Here's how the part is built. I have some questions about the finished solid (model axes, mm). A direction names the side the tool comes from. Give positions to 0.01 mm unless a question says otherwise; leave off trailing zeros. Write each loop counter-clockwise with the first axis right and the second up, starting at its lowest first coordinate (ties: lowest second). Pieces come first, ordered by that corner, then holes. Notation, with made-up numbers: (73, 46.25) - (94, 46.25) arc R22 cw to (94, 77.25) - close; hole circle Ø4 at (-34, 35.25). An arc over 180 degrees is marked (long way). Use a Markdown table: item, result.
```python
from build123d import *

# Parameters (mm, degrees)
PIVOT_HUB_SKETCH_R            = 28
PIVOT_HUB_SKETCH_R_2          = 15
PIVOT_HUB_56_BORE_30_DEPTH    = 40
LINK_ARM_DEPTH                = 24
FORK_SLOT_SKETCH_W            = 63.247521784
FORK_SLOT_SKETCH_H            = 16
FORK_SLOT_16_DEPTH            = 146.327216997
UPRIGHT_BOSS_SKETCH_R         = 16
UPRIGHT_BOSS_SKETCH_R_2       = 8
UPRIGHT_BOSS_32_BORE_16_DEPTH = 40
JUNCTION_PAD_REACH            = 171.706
TRIANGULAR_RELIEF_CUT_DEPTH   = 10


with BuildPart() as part:
    # Pivot Hub Sketch → Pivot Hub Ø56 Bore Ø30 (new, symmetric)
    with BuildSketch(Plane.XY):
        Circle(PIVOT_HUB_SKETCH_R)
        Circle(PIVOT_HUB_SKETCH_R_2, mode=Mode.SUBTRACT)
    extrude(amount=PIVOT_HUB_56_BORE_30_DEPTH, both=True)

    # Link Arm Profile → Link Arm (add, symmetric)
    with BuildSketch(Plane.XY):
        with BuildLine():
            Line((0, 28), (72, 28))
            ThreePointArc((72, 28), (77.656854249, 30.343145751), (80, 36))
            Line((80, 36), (128, 36))
            Line((128, 36), (128, -4))
            Line((128, -4), (100, -4))
            Line((100, -4), (100, 4))
            ThreePointArc((100, 4), (97.656854249, 9.656854249), (92, 12))
            Line((92, 12), (52, 12))
            ThreePointArc((52, 12), (46.343145751, 9.656854249), (44, 4))
            Line((44, 4), (44, -28))
            Line((44, -28), (0, -28))
            ThreePointArc((0, -28), (28, 0), (0, 28))
        make_face()
    extrude(amount=LINK_ARM_DEPTH, both=True)

    # Fork Slot Sketch → Fork Slot 16 (cut, through all)
    with BuildSketch(Plane(origin=(0, 28, 0), x_dir=(1, 0, 0), z_dir=(0, 1, 0))):
        with Locations((-3.623760892, 0)):
            Rectangle(FORK_SLOT_SKETCH_W, FORK_SLOT_SKETCH_H)
    extrude(amount=-FORK_SLOT_16_DEPTH, mode=Mode.SUBTRACT)

    # Upright Boss Sketch → Upright Boss Ø32 Bore Ø16 (add)
    with BuildSketch(Plane(origin=(0, 36, 0), x_dir=(1, 0, 0), z_dir=(0, 1, 0))):
        with Locations((103.942410132, 0)):
            Circle(UPRIGHT_BOSS_SKETCH_R)
        with Locations(Location((103.942410132, 0, 0), (0, 0, 180))):
            Circle(UPRIGHT_BOSS_SKETCH_R_2, mode=Mode.SUBTRACT)
    extrude(amount=UPRIGHT_BOSS_32_BORE_16_DEPTH)

    # Junction Pad Sketch → Junction Pad (add, up to next)
    with BuildSketch(Plane(origin=(0, 76, 0), x_dir=(1, 0, 0), z_dir=(0, 1, 0)), mode=Mode.PRIVATE) as junction_pad_sk1:
        with BuildLine():
            Line((48, 5), (88.743725978, 5))
            ThreePointArc((88.743725978, 5), (87.942410132, 0), (88.743725978, -5))
            Line((88.743725978, -5), (48, -5))
            Line((48, -5), (48, 5))
        make_face()
    junction_pad_tool1 = extrude(junction_pad_sk1.sketch, amount=-JUNCTION_PAD_REACH, mode=Mode.PRIVATE) - part.part
    add(junction_pad_tool1.solids().sort_by_distance((68.104095, 76, 0))[0])

    # Relief Cut Sketch → Triangular Relief Cut (cut)
    with BuildSketch(Plane.XY.offset(5)):
        Polygon((88.743725978, 76), (48, 28), (48, 76), align=None)
    extrude(amount=-TRIANGULAR_RELIEF_CUT_DEPTH, mode=Mode.SUBTRACT)


solid = part.part
```
Item 1: I need wall thicknesses on line 1 along X through (y, z) = (0, -18.5); line 2 along Y through (x, z) = (0, 17.5); line 3 along X through (y, z) = (18, 5). Which ranges of each line are inside material? Lowest first, please. Write a range as [from, to].
Values:
| item | result |
|---|---|
| line 1 | x = [-28, -15], [15, 44], [100, 128] |
| line 2 | y = [-28, -15], [15, 28] |
| line 3 | x = [28, 128] |
Item 2: If we section it at D-D, the plane x = 23: Write out the boundary of the cut face in (y, z).
Values:
| item | result |
|---|---|
| outline | (-28, -24) - (-15.97, -24) - (-15.97, -40) - (15.97, -40) - (15.97, -24) - (28, -24) - (28, -8) - (-28, -8) - close; (-28, 8) - (28, 8) - (28, 24) - (15.97, 24) - (15.97, 40) - (-15.97, 40) - (-15.97, 24) - (-28, 24) - close |
Item 3: For faces 1 (the flat face through (44, -12, 0)), 2 (the flat face through (12, -12, -8)), 3 (the cylindrical face through (-27.973, 1.231, 27.78)), which set-ups out of +Z, -Z, +X, -X, +Y, -Y let a thin tool reach every point of the face, with its end or its side?
Values:
| item | result |
|---|---|
| face 1 | +Z, -Z, -Y |
| face 2 | -X, +Y, -Y |
| face 3 | +Z |
Item 4: If we section it at C-C, the plane z = 0: Write out the boundary of the cut face in (x, y).
Values:
| item | result |
|---|---|
| outline | (28, -28) - (44, -28) - (44, 4) arc R8 cw to (52, 12) - (92, 12) arc R8 cw to (100, 4) - (100, -4) - (128, -4) - (128, 36) - (119.94, 36) - (119.94, 76) - (111.94, 76) - (111.94, 36) - (95.94, 36) - (95.94, 76) - (88.74, 76) - (48, 28) - (28, 28) - close |
Item 5: If we section it at A-A, the plane z = -18: Write out the boundary of the cut face in (x, y), plus the area to 3 significant figures.
Values:
| item | result |
|---|---|
| outline | (0, -28) - (44, -28) - (44, 4) arc R8 cw to (52, 12) - (92, 12) arc R8 cw to (100, 4) - (100, -4) - (128, -4) - (128, 36) - (80, 36) arc R8 cw to (72, 28) - (0, 28) arc R28 ccw to start; hole circle Ø30 at (0, 0) |
| area | 5,210 mm2 |
Item 6: Thinking about a two-plate mould opening in X: for faces 4 (the cylindrical face through (119.93, 55.72, 0.63)), 5 (the flat face through (12, -12, 8)), 6 (the cylindrical face through (97.719, 9.594, 0.336)), which applies, +X half, -X half, draft (parallel to the pull), parting line (faces both ways), or undercut?
Values:
| item | result |
|---|---|
| face 4 | parting line |
| face 5 | draft |
| face 6 | undercut |
Item 7: Will these pins go through, and if not, where does the flat tip stop? pin 1 Ø1 at (y, z) = (-17, 18) entering from -X; pin 2 Ø5 at (x, y) = (55.5, 15) entering from +Z; pin 3 Ø9 at (y, z) = (-1, 4.5) entering from -X.
Values:
| item | result |
|---|---|
| pin 1 | stops at x = -22.62 |
| pin 2 | stops at z = 24 |
| pin 3 | stops at x = -28 |
Item 8: If we section it at B-B, the plane y = 0: Write out the boundary of the cut face in (x, z).
Values:
| item | result |
|---|---|
| outline | (-28, -40) - (-15, -40) - (-15, -8) - (-28, -8) - close; (-28, 8) - (-15, 8) - (-15, 40) - (-28, 40) - close; (15, -40) - (28, -40) - (28, -24) - (44, -24) - (44, 24) - (28, 24) - (28, 40) - (15, 40) - (15, 8) - (28, 8) - (28, -8) - (15, -8) - close; (100, -24) - (128, -24) - (128, 24) - (100, 24) - close |
